The listing builds one solid part. Answer for the finished solid, in the listing's coordinates (mm). Face numbers are marked on the shaded views. A direction names the side the tool comes from. Coordinates: 2 decimals unless noted, no trailing zeros. Loops run counter-clockwise (first coordinate to the right, second up) from the corner with the lowest first, then second, coordinate; pieces in that order, holes last. Notation, with made-up numbers: (7, -6) -> (17, -6) arc R22 cw to (17, 24) -> close; hole circle Ø5 at (82.5, 72). An arc over 180 degrees is marked (long way). Answer in a Markdown table with one row per item.
```python
from build123d import *

# Parameters (mm, degrees)
SKETCH1_W                                           = 130
SKETCH1_H                                           = 95
BOSS_EXTRUDE1_DEPTH                                 = 15
CBORE_FOR_M8_HEX_SOCKET_HEAD_CAP_SCREW1_D           = 9
CBORE_FOR_M8_HEX_SOCKET_HEAD_CAP_SCREW1_CBORE_D     = 15
CBORE_FOR_M8_HEX_SOCKET_HEAD_CAP_SCREW1_CBORE_DEPTH = 8.6
CHAMFER1_SIZE                                       = 10
CBORE_FOR_M6_HEX_SOCKET_HEAD_CAP_SCREW1_D           = 6.6
CBORE_FOR_M6_HEX_SOCKET_HEAD_CAP_SCREW1_CBORE_D     = 11
CBORE_FOR_M6_HEX_SOCKET_HEAD_CAP_SCREW1_CBORE_DEPTH = 6.4


with BuildPart() as part:
    # Sketch1 → Boss-Extrude1 (new body)
    with BuildSketch(Plane.XY):
        Rectangle(SKETCH1_W, SKETCH1_H)
    extrude(amount=BOSS_EXTRUDE1_DEPTH)

    # CBORE for M8 Hex Socket Head Cap Screw1 (through all)
    with Locations(Plane.XY.offset(15)):
        with Locations((54, 27.5), (54, -27.5), (-54, 27.5), (-54, -27.5), (0, 27.5), (0, -27.5)):
            CounterBoreHole(CBORE_FOR_M8_HEX_SOCKET_HEAD_CAP_SCREW1_D / 2, CBORE_FOR_M8_HEX_SOCKET_HEAD_CAP_SCREW1_CBORE_D / 2, CBORE_FOR_M8_HEX_SOCKET_HEAD_CAP_SCREW1_CBORE_DEPTH)

    # Chamfer1
    chamfer1_edges = [part.edges().sort_by_distance(p)[0] for p in [
        (-65, 47.5, 7.5),
        (65, 47.5, 7.5),
    ]]
    chamfer(chamfer1_edges, length=CHAMFER1_SIZE)

    # CBORE for M6 Hex Socket Head Cap Screw1 (through all)
    with Locations(Plane(origin=(0, 0, 0), x_dir=(-1, 0, 0), z_dir=(0, 0, -1))):
        with Locations((-34, -32.5), (-34, 0), (-34, 32.5), (34, -32.5), (34, 0), (34, 32.5)):
            CounterBoreHole(CBORE_FOR_M6_HEX_SOCKET_HEAD_CAP_SCREW1_D / 2, CBORE_FOR_M6_HEX_SOCKET_HEAD_CAP_SCREW1_CBORE_D / 2, CBORE_FOR_M6_HEX_SOCKET_HEAD_CAP_SCREW1_CBORE_DEPTH)


solid = part.part
```
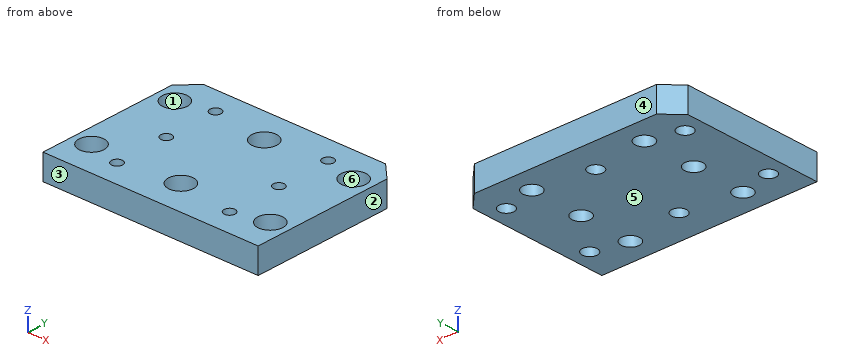
Item 1: A cutting plane is placed at D-D, the plane x = -34. Determine the outline of the cut face in (y, z), plus the area to 3 significant figures.
Findings below:
| item | result |
|---|---|
| outline | (-47.5, 0) -> (-38, 0) -> (-38, 6.4) -> (-35.8, 6.4) -> (-35.8, 15) -> (-47.5, 15) -> close; (-29.2, 6.4) -> (-27, 6.4) -> (-27, 0) -> (-5.5, 0) -> (-5.5, 6.4) -> (-3.3, 6.4) -> (-3.3, 15) -> (-29.2, 15) -> close; (3.3, 6.4) -> (5.5, 6.4) -> (5.5, 0) -> (27, 0) -> (27, 6.4) -> (29.2, 6.4) -> (29.2, 15) -> (3.3, 15) -> close; (35.8, 6.4) -> (38, 6.4) -> (38, 0) -> (47.5, 0) -> (47.5, 15) -> (35.8, 15) -> close |
| area | 1,040 mm2 |
Item 2: A tool of negligible diameter and unlimited length cuts with its end or side. For the marked faces 1 and 2, from which of +Z, -Z, +X, -X, +Y, -Y can it reach the whole face along a straight path? Write none if from no direction.
Findings below:
| item | result |
|---|---|
| face 1 | +Z |
| face 2 | +Z, -Z, +X, +Y, -Y |
Item 3: Flat-ended cylindrical pins translate along their axes: pin 1 Ø4.5 at (x, y) = (56.5, -29.5) entering from +Z; pin 2 Ø10.5 at (x, y) = (-34, 0) entering from -Z. Find the tip coordinate at first contact, or state that the pin passes through.
Findings below:
| item | result |
|---|---|
| pin 1 | stops at z = 6.4 |
| pin 2 | stops at z = 6.4 |
Item 4: Determine the mould class of the marked faces 3, 4, 5 and 6 for opening direction Y: +Y half, -Y half, draft (parallel to the pull), parting line (faces both ways), or undercut.
Findings below:
| item | result |
|---|---|
| face 3 | -Y half |
| face 4 | +Y half |
| face 5 | draft |
| face 6 | undercut |
Item 5: A cutting plane is placed at C-C, the plane y = 0. Determine the outline of the cut face in (x, z).
Findings below:
| item | result |
|---|---|
| outline | (-65, 0) -> (-39.5, 0) -> (-39.5, 6.4) -> (-37.3, 6.4) -> (-37.3, 15) -> (-65, 15) -> close; (-30.7, 6.4) -> (-28.5, 6.4) -> (-28.5, 0) -> (28.5, 0) -> (28.5, 6.4) -> (30.7, 6.4) -> (30.7, 15) -> (-30.7, 15) -> close; (37.3, 6.4) -> (39.5, 6.4) -> (39.5, 0) -> (65, 0) -> (65, 15) -> (37.3, 15) -> close |
Item 6: A cutting plane is placed at B-B, the plane z = 2.25. Count the separate pieces of the cut face and the enclosed holes in it, plus the area to 3 significant figures.
Findings below:
| item | result |
|---|---|
| separate pieces | 1 |
| enclosed holes | 12 |
| area | 11,300 mm2 |
Item 7: A cutting plane is placed at A-A, the plane x = 0. Determine the outline of the cut face in (y, z), plus the area to 3 significant figures.
Findings below:
| item | result |
|---|---|
| outline | (-47.5, 0) -> (-32, 0) -> (-32, 6.4) -> (-35, 6.4) -> (-35, 15) -> (-47.5, 15) -> close; (-23, 0) -> (23, 0) -> (23, 6.4) -> (20, 6.4) -> (20, 15) -> (-20, 15) -> (-20, 6.4) -> (-23, 6.4) -> close; (32, 0) -> (47.5, 0) -> (47.5, 15) -> (35, 15) -> (35, 6.4) -> (32, 6.4) -> close |
| area | 1,050 mm2 |
Item 8: Find the intervals of material crossed by probe 1 along Y at (x, z) = (0, 8.5); probe 2 along Y at (x, z) = (-34, 10.5); probe 3 along Y at (x, z) = (-34, 4), in increasing order.
Findings below:
| item | result |
|---|---|
| probe 1 | y = -47.5 to -35, -20 to 20, 35 to 47.5 |
| probe 2 | y = -47.5 to -35.8, -29.2 to -3.3, 3.3 to 29.2, 35.8 to 47.5 |
| probe 3 | y = -47.5 to -38, -27 to -5.5, 5.5 to 27, 38 to 47.5 |
